Could you check a few things on this model? Use its own coordinates, in mm. Coordinates: 2 decimals unless noted, no trailing zeros. Loops run counter-clockwise (first coordinate to the right, second up) from the corner with the lowest first, then second, coordinate; pieces in that order, holes last. Notation, with made-up numbers: (85.25, -16) -> (133.25, -16) arc R16 ccw to (133.25, -12) -> close; hole circle Ø7 at (31.5, 82.25). An arc over 180 degrees is marked (long way). One line per question, with ' | ' between items. Start each with the question number.
(1) Suppose I cut it at D-D (z = -6.75). Please give me the cut outline in (x, y).
(2) Suppose I cut it at A-A (z = -2.75). Please give me the cut outline in (x, y).
(3) If I drill on line 1 along Y through (x, z) = (10.5, -1.75); line 2 along X through (y, z) = (0.7, -3.5); line 3 along X through (y, z) = (0.2, -4.25), over which ranges is the centre line in solid material (lowest first)?
(4) I'm going to push flat-ended pins straight in: pin 1 Ø2.5 at (x, z) = (14, -3.5) entering from +Y; pin 2 Ø1 at (y, z) = (0.5, -6.5) entering from +X; pin 3 Ø1.5 at (y, z) = (1.5, -6.5) entering from +X. Where does each tip first touch, or does it pass through?
(5) Suppose I cut it at B-B (y = 1.55). Please give me the cut outline in (x, z), plus the area to 3 significant figures.
(6) Suppose I cut it at C-C (x = 9). Please give me the cut outline in (y, z), plus the area to 3 significant figures.
```python
from build123d import *

# Parameters (mm, degrees)
SKETCH1_W           = 33
SKETCH1_H           = 8
BOSS_EXTRUDE1_DEPTH = 2
SKETCH2_R           = 2.25
CUT_EXTRUDE1_DEPTH  = 25.560457127
SKETCH3_R           = 2
BOSS_EXTRUDE2_DEPTH = 1
CHAMFER2_SIZE       = 2


with BuildPart() as part:
    # Sketch1 → Boss-Extrude1 (new body)
    with BuildSketch(Plane(origin=(0, 0, 0), x_dir=(1, 0, 0), z_dir=(0, 1, 0))):
        with Locations((6.806648575, 3.484396201)):
            Rectangle(SKETCH1_W, SKETCH1_H)
    extrude(amount=BOSS_EXTRUDE1_DEPTH)

    # Sketch2 → Cut-Extrude1 (cut, through all)
    with BuildSketch(Plane(origin=(0, 2, 0), x_dir=(1, 0, 0), z_dir=(0, 1, 0))):
        with Locations(Location((-4.693351425, 3.484396201, 0), (0, 0, 270))):
            Circle(SKETCH2_R)
    extrude(amount=-CUT_EXTRUDE1_DEPTH, mode=Mode.SUBTRACT)

    # Sketch3 → Boss-Extrude2 (add)
    with BuildSketch(Plane(origin=(0, 2, 0), x_dir=(1, 0, 0), z_dir=(0, 1, 0))):
        with Locations(Location((19.306648575, 3.484396201, 0), (0, 0, 270))):
            Circle(SKETCH3_R)
    extrude(amount=BOSS_EXTRUDE2_DEPTH)

    # Chamfer2
    chamfer2_edges = [part.edges().sort_by_distance(p)[0] for p in [
        (-9.693351425, 1, -7.484396201),
        (23.306648575, 1, -7.484396201),
        (23.306648575, 1, 0.515603799),
        (-9.693351425, 1, 0.515603799),
    ]]
    chamfer(chamfer2_edges, length=CHAMFER2_SIZE)


solid = part.part
```
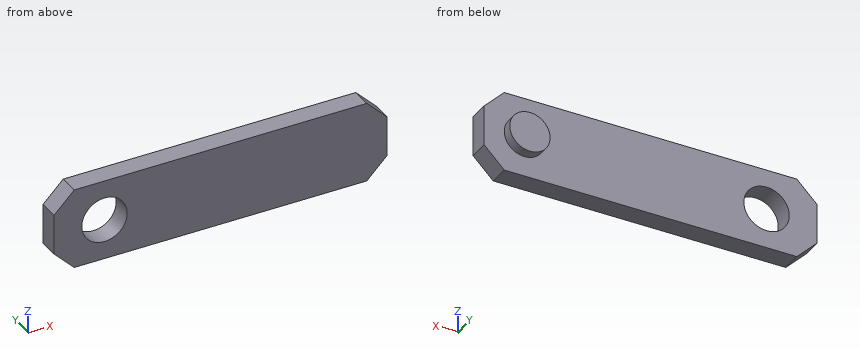
Checks:
1) outline: (-8.43, 0) -> (22.04, 0) -> (22.04, 2) -> (-8.43, 2) -> close
2) outline: (-9.69, 0) -> (-6.82, 0) -> (-6.82, 2) -> (-9.69, 2) -> close; (-2.57, 0) -> (23.31, 0) -> (23.31, 2) -> (21.17, 2) -> (21.17, 3) -> (17.45, 3) -> (17.45, 2) -> (-2.57, 2) -> close
3) line 1: y = 0 to 2 | line 2: x = -9.69 to -6.94, -2.44 to 23.31 | line 3: x = -9.69 to -6.81, -2.58 to 23.31
4) pin 1: stops at y = 2 | pin 2: stops at x = 22.79 | pin 3: stops at x = 23.04
5) outline: (-9.69, -5.48) -> (-7.69, -7.48) -> (21.31, -7.48) -> (23.31, -5.48) -> (23.31, -1.48) -> (21.31, 0.52) -> (-7.69, 0.52) -> (-9.69, -1.48) -> close; hole circle Ø4.5 at (-4.69, -3.48) | area: 240 mm^2
6) outline: (0, -7.48) -> (2, -7.48) -> (2, 0.52) -> (0, 0.52) -> close | area: 16.0 mm^2
